Geometry check sheet. Reference: the model listing, model coordinates, mm. Round coordinates to 2 decimals unless told otherwise and drop trailing zeros. Loops run counter-clockwise (first coordinate to the right, second up) from the corner with the lowest first, then second, coordinate; pieces in that order, holes last. Notation, with made-up numbers: (46.25, 66.5) -> (58.25, 66.5) arc R11 cw to (58.25, 73.5) -> close; hole circle Ø4 at (-3.75, -17.5). An arc over 180 degrees is marked (long way). Use a Markdown table: item, result. Add a question column.
Q1. Material ranges on L1, parallel to X at y = 1.5, z = 6; L2, parallel to Y at x = -12, z = 5.75; L3, parallel to Z at x = -2, y = -4.5, recorded low to high.
Q2. Gauge pin test, flat ends, axial feed: P1, Ø2, axis at y = -2, z = 4.5, coming from the +X side; P2, Ø3, axis at y = 4, z = 3, coming from the +X side. Record the tip position at first contact, or that the pin passes through.
Q3. Sectioned sample at A-A, the plane z = 1.25. Enter the section's corners in (x, y).
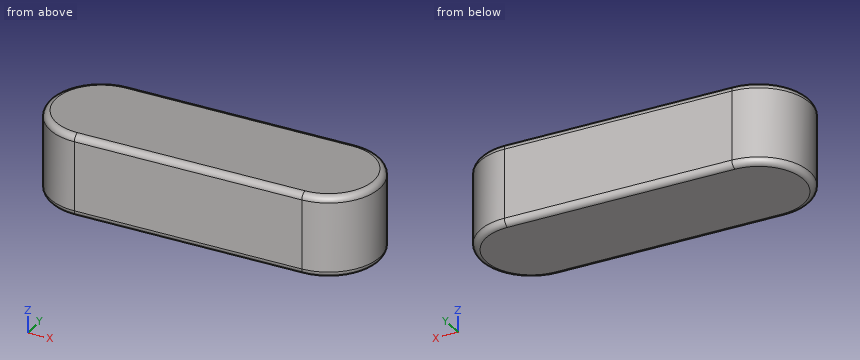
```python
from build123d import *

# Parameters (mm, degrees)
EXTRUDE_523_DEPTH = 8
FILLET_1_R        = 0.6


with BuildPart() as part:
    # 草图1 → Extrude 523 (new body)
    with BuildSketch(Plane.XY):
        with BuildLine():
            Line((-11, 5), (11, 5))
            ThreePointArc((11, 5), (16, 0), (11, -5))
            Line((11, -5), (-11, -5))
            ThreePointArc((-11, -5), (-16, 0), (-11, 5))
        make_face()
    extrude(amount=EXTRUDE_523_DEPTH)

    # 圆角1
    fillet_1_edges = [part.edges().sort_by_distance(p)[0] for p in [
        (16, 0, 8),
        (0, 5, 8),
        (-16, 0, 8),
        (0, 5, 0),
        (16, 0, 0),
        (0, -5, 0),
        (-16, 0, 0),
        (0, -5, 8),
    ]]
    fillet(fillet_1_edges, radius=FILLET_1_R)


solid = part.part
```
Values:
| question | item | result |
|---|---|---|
| 1 | L1 | -15.77 to 15.77 |
| 1 | L2 | -4.9 to 4.9 |
| 1 | L3 | 0.01 to 7.99 |
| 2 | P1 | x = 15.9 |
| 2 | P2 | x = 15.33 |
| 3 | outline | (-11, -5) -> (11, -5) arc R5 ccw to (11, 5) -> (-11, 5) arc R5 ccw to start |
